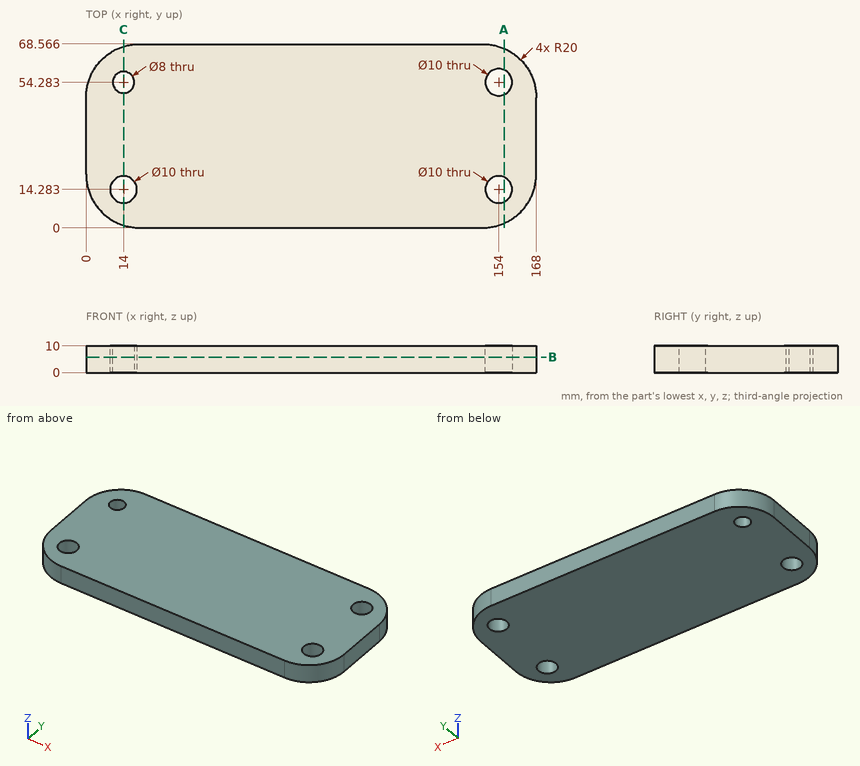
Could you check a few things on this drawing? It's one solid part, dimensions in mm from its lowest x, y, z. Coordinates: 2 decimals unless noted, no trailing zeros. Write each loop counter-clockwise with the first axis right and the second up, starting at its lowest first coordinate (ties: lowest second). Pieces come first, ordered by that corner, then holes. Notation, with made-up numbers: (-26, 70) - (-3, 70) arc R17 ccw to (-3, 77) - close; hole circle Ø10 at (-9.5, -7.5). An arc over 180 degrees is marked (long way). Put each result on its own line as item: value. Start each with the question number.
Q1. I want a section at C-C on x = 14. Write out the boundary of the cut face in (y, z) (1 decimal).
Q2. I want a section at A-A on x = 156. Write out the boundary of the cut face in (y, z) (1 decimal), plus the area to 3 significant figures.
Q3. Please list where these lines run through material, in increasing order: L1, parallel to X at y = 10, z = 6; L2, parallel to X at y = 13.5, z = 4.75 (1 decimal); L3, parallel to X at y = 19.5, z = 7.75.
Q4. I want a section at B-B on z = 5.75. Write out the boundary of the cut face in (x, y), plus the area to 3 significant figures.
Checks:
1. outline: (0.9, 0) - (9.3, 0) - (9.3, 10) - (0.9, 10) - close; (19.3, 0) - (50.3, 0) - (50.3, 10) - (19.3, 10) - close; (58.3, 0) - (67.6, 0) - (67.6, 10) - (58.3, 10) - close
2. outline: (1.7, 0) - (9.7, 0) - (9.7, 10) - (1.7, 10) - close; (18.9, 0) - (49.7, 0) - (49.7, 10) - (18.9, 10) - close; (58.9, 0) - (66.9, 0) - (66.9, 10) - (58.9, 10) - close
2. area: 469 mm²
3. L1: 2.68 to 11.42, 16.58 to 151.42, 156.58 to 165.32
3. L2: 1.1 to 9.1, 18.9 to 149.1, 158.9 to 166.9
3. L3: 0.01 to 167.99
4. outline: (0, 20) arc R20 ccw to (20, 0) - (148, 0) arc R20 ccw to (168, 20) - (168, 48.57) arc R20 ccw to (148, 68.57) - (20, 68.57) arc R20 ccw to (0, 48.57) - close; hole circle Ø10 at (14, 14.28); hole circle Ø8 at (14, 54.28); hole circle Ø10 at (154, 14.28); hole circle Ø10 at (154, 54.28)
4. area: 10,900 mm²
